Could you check a few things on this model? Use its own coordinates, in mm. Give positions to 0.01 mm unless a question says otherwise; leave off trailing zeros. Order: outer loops, then holes, each group sorted by start corner. A loop starts at its lowest first (then second) coordinate and runs counter-clockwise, first axis right, second up. Notation, with made-up numbers: (35.5, 9) -> (46.5, 9) arc R22 ccw to (46.5, 47) -> close; hole circle Ø7 at (55.5, 36). An arc over 180 degrees is marked (long way). One line per item, written item: value.
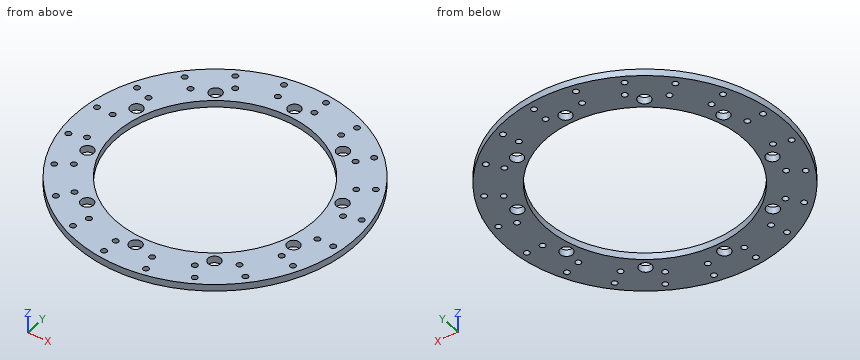
```python
from build123d import *

# Parameters (mm, degrees)
SKETCH_1_R               = 61.5
SKETCH_1_R_2             = 43.5
EXTRUDE_1_DEPTH          = 1.5
HOLE_WIZARD_5_5_5_5_2_D  = 5.5
HOLE_WIZARD_M3_1_D       = 2.5
PATTERN_CIRCULAR_1_COUNT = 10
PATTERN_CIRCULAR_2_COUNT = 20


with BuildPart() as part:
    # 草图1 → 凸台-拉伸1 (new, symmetric)
    with BuildSketch(Plane.XY):
        Circle(SKETCH_1_R)
        Circle(SKETCH_1_R_2, mode=Mode.SUBTRACT)
    extrude(amount=EXTRUDE_1_DEPTH, both=True)

    # Ø5.5 (5.5) 直径孔2 (through all)
    with Locations(Plane.XY.offset(1.5)):
        with Locations((0, 48)):
            hole_wizard_5_5_5_5_2 = Hole(HOLE_WIZARD_5_5_5_5_2_D / 2)

    # M3 螺纹孔1 (through all)
    with Locations(Plane.XY.offset(1.5)):
        with Locations((-57.5, 7), (-50.5, 7)):
            hole_wizard_m3_1 = Hole(HOLE_WIZARD_M3_1_D / 2)

    # 阵列(圆周)1: Ø5.5 (5.5) 直径孔2 ×10 about axis
    pattern_circular_1_axis = Axis((0, 0, 0), (0, 0, 1))
    for i in range(1, PATTERN_CIRCULAR_1_COUNT):
        add(hole_wizard_5_5_5_5_2.rotate(pattern_circular_1_axis, i * 360 / PATTERN_CIRCULAR_1_COUNT), mode=Mode.SUBTRACT)

    # 阵列(圆周)2: M3 螺纹孔1 ×20 about axis
    pattern_circular_2_axis = Axis((0, 0, 0), (0, 0, 1))
    for i in range(1, PATTERN_CIRCULAR_2_COUNT):
        add(hole_wizard_m3_1.rotate(pattern_circular_2_axis, i * 360 / PATTERN_CIRCULAR_2_COUNT), mode=Mode.SUBTRACT)


solid = part.part
```
1) For P1, Ø2, axis at x = 28.13, y = -50.63, coming from the +Z side; P2, Ø3, axis at x = -52.52, y = 24.43, coming from the -Z side; P3, Ø1.5, axis at y = 22.5, z = -1, coming from the -X side, each with a flat end and sliding along its axis, tell me the tip position at first contact or that it passes through.
Answer below:
P1: passes through
P2: stops at z = -1.5
P3: stops at x = -57.53
2) Suppose I cut it at B-B, the plane y = 19.5. Write out the boundary of the cut face in (x, z), then the cut area to 3 significant figures.
Answer below:
outline: (-58.33, -1.5) -> (-38.88, -1.5) -> (-38.88, 1.5) -> (-58.33, 1.5) -> close; (38.88, -1.5) -> (58.33, -1.5) -> (58.33, 1.5) -> (38.88, 1.5) -> close
area: 117 mm2
3) Suppose I cut it at C-C, the plane z = 0.9. State how many separate pieces and enclosed holes the cut face has, then the cut area to 3 significant figures.
Answer below:
separate pieces: 1
enclosed holes: 51
area: 5,500 mm2
4) Suppose I cut it at A-A, the plane x = 0. Write out the boundary of the cut face in (y, z), then the cut area to 3 significant figures.
Answer below:
outline: (-61.5, -1.5) -> (-50.75, -1.5) -> (-50.75, 1.5) -> (-61.5, 1.5) -> close; (-45.25, -1.5) -> (-43.5, -1.5) -> (-43.5, 1.5) -> (-45.25, 1.5) -> close; (43.5, -1.5) -> (45.25, -1.5) -> (45.25, 1.5) -> (43.5, 1.5) -> close; (50.75, -1.5) -> (61.5, -1.5) -> (61.5, 1.5) -> (50.75, 1.5) -> close
area: 75.0 mm2
5) If I drill on line 1 along Y through (x, z) = (0, -0.45); line 2 along Y through (x, z) = (-50.5, 0.75); line 3 along Y through (x, z) = (-37.5, -0.75), over which ranges is the centre line in solid material (lowest first)?
Answer below:
line 1: y = -61.5 to -50.75, -45.25 to -43.5, 43.5 to 45.25, 50.75 to 61.5
line 2: y = -35.1 to -29.38, -26.89 to -10.16, -7.74 to 5.75, 8.25 to 35.1
line 3: y = -48.74 to -22.05, 22.05 to 34.35, 36.34 to 48.74
